Verification items for the finished model (mm, model axes). A direction names the side the tool comes from. Round coordinates to 2 decimals unless told otherwise and drop trailing zeros. Write each loop counter-clockwise with the first axis right and the second up, starting at its lowest first coordinate (ties: lowest second). Pieces come first, ordered by that corner, then holes.
from build123d import *

# Parameters (mm, degrees)
SKETCH1_R           = 17
BOSS_EXTRUDE1_DEPTH = 4
CUT_EXTRUDE1_DEPTH  = 3
SKETCH3_R           = 2
CUT_EXTRUDE2_DEPTH  = 4
CUT_EXTRUDE3_DEPTH  = 3
SKETCH7_R           = 1.5
BOSS_EXTRUDE3_DEPTH = 2


with BuildPart() as part:
    # Sketch1 → Boss-Extrude1 (new body)
    with BuildSketch(Plane.XY):
        Circle(SKETCH1_R)
    extrude(amount=BOSS_EXTRUDE1_DEPTH)

    # Sketch2 → Cut-Extrude1 (cut)
    with BuildSketch(Plane.XY.offset(4)):
        with BuildLine():
            ThreePointArc((9.192388155, 9.192388155), (0, 13), (-9.192388155, 9.192388155))
            ThreePointArc((-9.192388155, 9.192388155), (-9.192388155, 6.363961031), (-6.363961031, 6.363961031))
            ThreePointArc((-6.363961031, 6.363961031), (0, 9), (6.363961031, 6.363961031))
            ThreePointArc((6.363961031, 6.363961031), (9.192388155, 6.363961031), (9.192388155, 9.192388155))
        make_face()
    extrude(amount=-CUT_EXTRUDE1_DEPTH, mode=Mode.SUBTRACT)

    # Sketch3 → Cut-Extrude2 (cut)
    with BuildSketch(Plane.XY.offset(4)):
        with Locations((7.778174593, 7.778174593)):
            Circle(SKETCH3_R)
        with Locations((-7.778174593, 7.778174593)):
            Circle(SKETCH3_R)
    extrude(amount=-CUT_EXTRUDE2_DEPTH, mode=Mode.SUBTRACT)

    # Sketch4 → Cut-Extrude3 (cut)
    with BuildSketch(Plane.XY.offset(4)):
        with BuildLine():
            ThreePointArc((-9.192388155, -9.192388155), (0, -13), (9.192388155, -9.192388155))
            ThreePointArc((9.192388155, -9.192388155), (9.192388155, -6.363961031), (6.363961031, -6.363961031))
            ThreePointArc((6.363961031, -6.363961031), (0, -9), (-6.363961031, -6.363961031))
            ThreePointArc((-6.363961031, -6.363961031), (-9.192388155, -6.363961031), (-9.192388155, -9.192388155))
        make_face()
    extrude(amount=-CUT_EXTRUDE3_DEPTH, mode=Mode.SUBTRACT)

    # Sketch7 → Boss-Extrude3 (add)
    with BuildSketch(Plane(origin=(0, 0, 0), x_dir=(-1, 0, 0), z_dir=(0, 0, -1))):
        with Locations(Location((11, 0, 0), (0, 0, 180))):
            Circle(SKETCH7_R)
        with Locations(Location((-11, 0, 0), (0, 0, 180))):
            Circle(SKETCH7_R)
    extrude(amount=BOSS_EXTRUDE3_DEPTH)


solid = part.part
Q1. Tool access check on faces 4 (the cylindrical face through (-12.5, -0.07, -0.99)), 5 (the cylindrical face through (0, -9, 3)), 6 (the cylindrical face through (-9.365, 6.561, 1.584)). Record the directions out of +Z, -Z, +X, -X, +Y, -Y that give a thin tool (end or side, any length) a straight path to the whole face; none if there is none.
Recorded:
face 4: -Z
face 5: +Z
face 6: +Z, -Z
Q2. Sectioned sample at A-A (x = 0). Enter the section's corners in (y, z).
Recorded:
outline: (-17, 0) - (17, 0) - (17, 4) - (13, 4) - (13, 1) - (9, 1) - (9, 4) - (-9, 4) - (-9, 1) - (-13, 1) - (-13, 4) - (-17, 4) - close
Q3. Release check for a two-part mould opening along Y. For faces 1 (the flat face through (0, 0, 0)), 2 (the cylindrical face through (9.5, -0.07, -0.99)), 3 (the cylindrical face through (0, 9, 3)) record: released by +Y, released by -Y, zero draft, split by the parting line, or undercut.
Recorded:
face 1: zero draft
face 2: split by the parting line
face 3: undercut
Q4. Material ranges on line 1 along Y through (x, z) = (7.5, 3.2); line 2 along Y through (x, z) = (9, 1.8); line 3 along X through (y, z) = (-6, 2.9), recorded low to high.
Recorded:
line 1: y = -15.26 to -10.62, -5.8 to 5.8, 10.62 to 15.26
line 2: y = -14.42 to -9.38, -6.19 to 6.19, 9.38 to 14.42
line 3: x = -15.91 to -8.69, -6.86 to 6.86, 8.69 to 15.91
Q5. Sectioned sample at B-B (y = 0). Enter the section's corners in (x, z).
Recorded:
outline: (-17, 0) - (-12.5, 0) - (-12.5, -2) - (-9.5, -2) - (-9.5, 0) - (9.5, 0) - (9.5, -2) - (12.5, -2) - (12.5, 0) - (17, 0) - (17, 4) - (-17, 4) - close
Q6. Sectioned sample at C-C (z = 1.75). Enter the section's corners in (x, y), plus the area to 3 significant figures.
Recorded:
outline: circle Ø34 at (0, 0); hole (-9.19, -9.19) arc R13 ccw to (9.19, -9.19) arc R2 ccw to (6.36, -6.36) arc R9 cw to (-6.36, -6.36) arc R2 ccw to start; hole (-9.19, 9.19) arc R2 ccw to (-6.36, 6.36) arc R9 cw to (6.36, 6.36) arc R2 ccw to (9.19, 9.19) arc R13 ccw to start
area: 745 mm2
Q7. Sectioned sample at D-D (y = 8.5). Enter the section's corners in (x, z), plus the area to 3 significant figures.
Recorded:
outline: (-14.72, 0) - (-9.64, 0) - (-9.64, 4) - (-14.72, 4) - close; (-5.91, 0) - (5.91, 0) - (5.91, 1) - (2.96, 1) - (2.96, 4) - (-2.96, 4) - (-2.96, 1) - (-5.91, 1) - close; (9.64, 0) - (14.72, 0) - (14.72, 4) - (9.64, 4) - close
area: 70.2 mm2
Q8. Depth check by flat-ended pin: P1, Ø1, axis at x = -12.5, y = -12, coming from the -Z side; P2, Ø3, axis at x = 5, z = -0.5, coming from the +Y side; P3, Ø1.5, axis at x = 9, z = -0.5, coming from the -Y side. Enter the tip coordinate at first touch or a pass-through.
Recorded:
P1: stops at z = 0
P2: stops at y = 16.62
P3: stops at y = -14.76
